from build123d import *

# Parameters (mm, degrees)
SKETCH1_W                                  = 150
SKETCH1_H                                  = 40
BOSS_EXTRUDE1_DEPTH                        = 10
FILLET1_R                                  = 5
SOCKET_BUTTON_HEAD_SCREW_HOLE1_D           = 9
SOCKET_BUTTON_HEAD_SCREW_HOLE1_DEPTH       = 19.75
SOCKET_BUTTON_HEAD_SCREW_HOLE1_CSINK_D     = 17.6
SOCKET_BUTTON_HEAD_SCREW_HOLE1_CSINK_ANGLE = 90
SOCKET_BUTTON_HEAD_SCREW_HOLE1_TIP         = 2.703872786


with BuildPart() as part:
    # Sketch1 → Boss-Extrude1 (new body)
    with BuildSketch(Plane(origin=(0, 0, 0), x_dir=(1, 0, 0), z_dir=(0, 1, 0))):
        with Locations((75, 20)):
            Rectangle(SKETCH1_W, SKETCH1_H)
    extrude(amount=BOSS_EXTRUDE1_DEPTH)

    # Fillet1
    fillet1_edges = [part.edges().sort_by_distance(p)[0] for p in [
        (0, 5, -40),
        (150, 5, -40),
        (150, 5, 0),
        (0, 5, 0),
    ]]
    fillet(fillet1_edges, radius=FILLET1_R)

    # Socket Button Head Screw Hole1
    with Locations(Plane(origin=(0, 10, 0), x_dir=(1, 0, 0), z_dir=(0, 1, 0))):
        with Locations((75, 20), (15, 20), (135, 20)):
            CounterSinkHole(SOCKET_BUTTON_HEAD_SCREW_HOLE1_D / 2, SOCKET_BUTTON_HEAD_SCREW_HOLE1_CSINK_D / 2, depth=SOCKET_BUTTON_HEAD_SCREW_HOLE1_DEPTH, counter_sink_angle=SOCKET_BUTTON_HEAD_SCREW_HOLE1_CSINK_ANGLE)
            with Locations((0, 0, -(SOCKET_BUTTON_HEAD_SCREW_HOLE1_DEPTH + SOCKET_BUTTON_HEAD_SCREW_HOLE1_TIP / 2))):  # 118° drill point
                Cone(0, SOCKET_BUTTON_HEAD_SCREW_HOLE1_D / 2, SOCKET_BUTTON_HEAD_SCREW_HOLE1_TIP, mode=Mode.SUBTRACT)


solid = part.part
Build history of the part. All positions in model axes, mm. Round coordinates to 2 decimals unless told otherwise and drop trailing zeros. Order: outer loops, then holes, each group sorted by start corner. A loop starts at its lowest first (then second) coordinate and runs counter-clockwise, first axis right, second up. Notation, with made-up numbers: M 0.5,13 L 35.5,13 A28 cw 35.5,39 Z; hole C -9.75,22 d1. An arc over 180 degrees is marked long. Use CSV: the item, a comma, the result in double quotes. Start each with the question number.
(1) Cut at A-A on x = 75. List the corners of the cut face in (y, z).
(2) Cut at C-C on y = 1.5. List the corners of the cut face in (x, z), then the cut area to 3 significant figures.
(3) Cut at B-B on z = -20. List the corners of the cut face in (x, y).
(4) Flat gauge pins, fed straight in: P1, Ø11.5, axis at x = 135, z = -20, coming from the +Y side; P2, Ø14.5, axis at x = 15, z = -20, coming from the +Y side. Where does each tip first touch, or does it go through?
(5) Mould opens along X. For faces 1 (the face through (72.581, 2.81, -23.794)), 2 (the face through (150, 5, -20)), 3 (the face through (74, 5, -40)) say: +X half, -X half, draft (parallel to the pull), parting line (faces both ways), or undercut.
(6) Drill centre lines: probe 1 along X at (y, z) = (1.3, -20); probe 2 along X at (y, z) = (7, -19.5); probe 3 along Z at (x, y) = (15, 1.3). Where is each one in solid material? Low to high.
Findings:
1,outline,"M 0,-40 L 10,-40 L 10,-28.8 L 5.7,-24.5 L 0,-24.5 Z; M 0,-15.5 L 5.7,-15.5 L 10,-11.2 L 10,0 L 0,0 Z"
2,outline,"M 0,-35 A5 ccw 5,-40 L 145,-40 A5 ccw 150,-35 L 150,-5 A5 ccw 145,0 L 5,0 A5 ccw 0,-5 Z; hole C 15,-20 d9; hole C 75,-20 d9; hole C 135,-20 d9"
2,area,"5,790 mm^2"
3,outline,"M 0,0 L 10.5,0 L 10.5,5.7 L 6.2,10 L 0,10 Z; M 19.5,0 L 70.5,0 L 70.5,5.7 L 66.2,10 L 23.8,10 L 19.5,5.7 Z; M 79.5,0 L 130.5,0 L 130.5,5.7 L 126.2,10 L 83.8,10 L 79.5,5.7 Z; M 139.5,0 L 150,0 L 150,10 L 143.8,10 L 139.5,5.7 Z"
4,P1,"stops at y = 6.95"
4,P2,"stops at y = 8.45"
5,face 1,"undercut"
5,face 2,"+X half"
5,face 3,"draft"
6,probe 1,"x = 0 to 10.5, 19.5 to 70.5, 79.5 to 130.5, 139.5 to 150"
6,probe 2,"x = 0 to 9.22, 20.78 to 69.22, 80.78 to 129.22, 140.78 to 150"
6,probe 3,"z = -40 to -24.5, -15.5 to 0"
